Verification items for this drawing (mm, ordinates from the low corner). Give positions to 0.01 mm unless a question says otherwise; leave off trailing zeros. Write each loop counter-clockwise with the first axis right and the second up, starting at its lowest first coordinate (ties: lowest second). Pieces come first, ordered by that corner, then holes. Notation, with made-up numbers: M 31,60 L 57,60 A27 ccw 57,85 Z; hole C 80,9.5 d2. An arc over 180 degrees is marked long. Use one line per item in the form item = value. Start each with the question number.
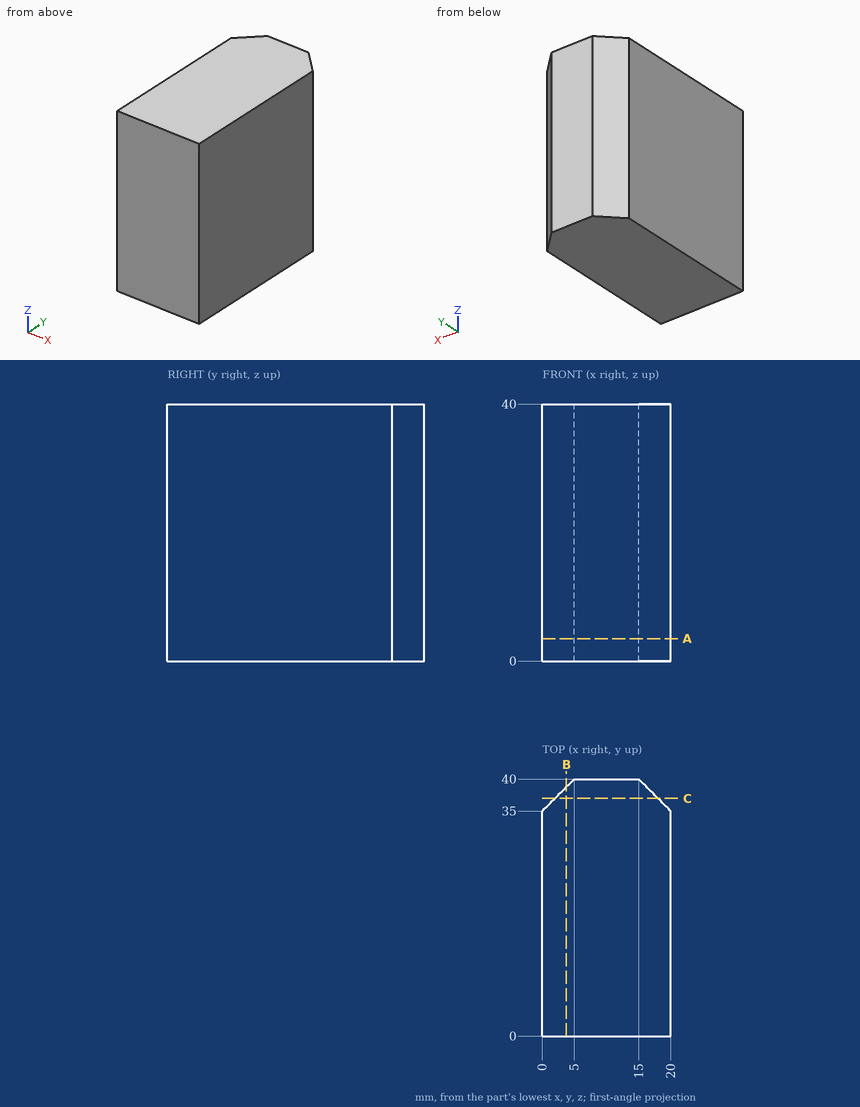
(1) Sectioned sample at A-A, the plane z = 3.5. Record the boundary of the cut face in (x, y), plus the area to 3 significant figures.
(2) Sectioned sample at C-C, the plane y = 37. Record the boundary of the cut face in (x, z), plus the area to 3 significant figures.
(3) Thickness scan on probe 1 along Y at (x, z) = (17.25, 30.5); probe 2 along Y at (x, z) = (3.5, 6); probe 3 along X at (y, z) = (37.5, 28). Record the ranges inside material, lowest first. Write a range as [from, to].
(4) Sectioned sample at B-B, the plane x = 3.75. Record the boundary of the cut face in (y, z).
Numbers:
q1.outline = M 0,0 L 20,0 L 20,35 L 15,40 L 5,40 L 0,35 Z
q1.area = 775 mm2
q2.outline = M 2,0 L 18,0 L 18,40 L 2,40 Z
q2.area = 640 mm2
q3.probe_1 = [0, 37.75]
q3.probe_2 = [0, 38.5]
q3.probe_3 = [2.5, 17.5]
q4.outline = M 0,0 L 38.75,0 L 38.75,40 L 0,40 Z
